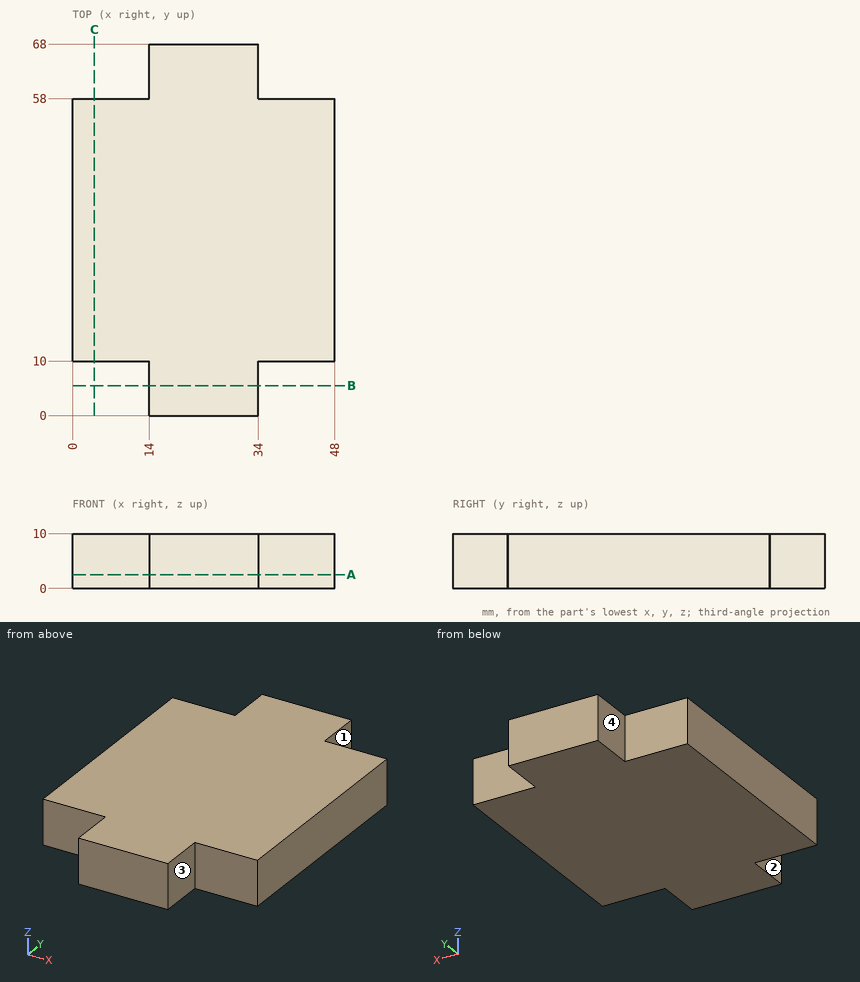
Part print with two shaded views. Sizes in mm from the minimum x, y, z corner. A direction names the side the tool comes from. Give positions to 0.01 mm unless a question says otherwise; leave off trailing zeros. Loops run counter-clockwise (first coordinate to the right, second up) from the corner with the lowest first, then second, coordinate; pieces in that order, holes last. Notation, with made-up numbers: (77.25, -3.5) -> (110.25, -3.5) arc R19 cw to (110.25, 3.5) -> close; hole circle Ø2 at (16, 53). An arc over 180 degrees is marked (long way). One line per question, with ' | ' between items.
Q1. Drop flat-ended pins along their axis: pin 1 (5 mm diameter, centred on y = 2.5, z = 6.5, fed in from +X); pin 2 (5 mm diameter, centred on y = 7, z = 5, fed in from -X); pin 3 (5 mm diameter, centred on x = 7.5, z = 7.5, fed in from +Y). Give the stop position or say it passes through.
Filled sheet:
pin 1: stops at x = 34 | pin 2: stops at x = 14 | pin 3: stops at y = 58
Q2. Cut at A-A, the plane z = 2.5. Write the cut outline in (x, y), plus the area to 3 significant figures.
Filled sheet:
outline: (0, 10) -> (14, 10) -> (14, 0) -> (34, 0) -> (34, 10) -> (48, 10) -> (48, 58) -> (34, 58) -> (34, 68) -> (14, 68) -> (14, 58) -> (0, 58) -> close | area: 2,700 mm²
Q3. Cut at B-B, the plane y = 5.5. Write the cut outline in (x, z), plus the area to 3 significant figures.
Filled sheet:
outline: (14, 0) -> (34, 0) -> (34, 10) -> (14, 10) -> close | area: 200 mm²
Q4. Tool access for the marked faces 1, 2, 3 and 4: list every direction of +Z, -Z, +X, -X, +Y, -Y with a clear straight run to the whole face (end or side of a thin tool).
Filled sheet:
face 1: +Z, -Z, +X, +Y | face 2: +Z, -Z, -X, -Y | face 3: +Z, -Z, +X, -Y | face 4: +Z, -Z, -X, +Y
Q5. Drill centre lines: line 1 along X through (y, z) = (64, 5.5); line 2 along Y through (x, z) = (8, 1.5). Where is each one in solid material? Low to high. Write a range as [from, to].
Filled sheet:
line 1: x = [14, 34] | line 2: y = [10, 58]
Q6. Cut at C-C, the plane x = 4. Write the cut outline in (y, z).
Filled sheet:
outline: (10, 0) -> (58, 0) -> (58, 10) -> (10, 10) -> close
